The model under review builds one solid part; all positions refer to its coordinate system, in mm. A direction names the side the tool comes from. Coordinates: 2 decimals unless noted, no trailing zeros. Write each loop counter-clockwise with the first axis right and the second up, starting at its lowest first coordinate (ties: lowest second). Pieces come first, ordered by that corner, then holes.
```python
from build123d import *

# Parameters (mm, degrees)
BOSS_EXTRUDE1_DEPTH     = 2000
CUT_EXTRUDE1_DEPTH      = 2002.124683772
CUT_EXTRUDE1_DEPTH_BACK = 2002.124683772


with BuildPart() as part:
    # Sketch1 → Boss-Extrude1 (new body)
    with BuildSketch(Plane(origin=(0, 0, 0), x_dir=(1, 0, 0), z_dir=(0, 1, 0))):
        with BuildLine():
            Line((-20, -30), (20, -30))
            ThreePointArc((20, -30), (27.071067812, -27.071067812), (30, -20))
            Line((30, -20), (30, 20))
            ThreePointArc((30, 20), (27.071067812, 27.071067812), (20, 30))
            Line((20, 30), (-20, 30))
            ThreePointArc((-20, 30), (-27.071067812, 27.071067812), (-30, 20))
            Line((-30, 20), (-30, -20))
            ThreePointArc((-30, -20), (-27.071067812, -27.071067812), (-20, -30))
        make_face()
        with BuildLine():
            Line((-26, -20), (-26, 20))
            ThreePointArc((-26, 20), (-24.242640687, 24.242640687), (-20, 26))
            Line((-20, 26), (20, 26))
            ThreePointArc((20, 26), (24.242640687, 24.242640687), (26, 20))
            Line((26, 20), (26, -20))
            ThreePointArc((26, -20), (24.242640687, -24.242640687), (20, -26))
            Line((20, -26), (-20, -26))
            ThreePointArc((-20, -26), (-24.242640687, -24.242640687), (-26, -20))
        make_face(mode=Mode.SUBTRACT)
    extrude(amount=BOSS_EXTRUDE1_DEPTH)

    # Sketch2 → Cut-Extrude1 (cut, two sides: drawn at the far end of the back side and taken through both)
    with BuildSketch(Plane.XY.offset(30).offset(-CUT_EXTRUDE1_DEPTH_BACK)):
        Polygon((30, 0), (-30, 75.027298751), (-170.24369385, -210.007574385), align=None)
        Polygon((-30, 1484.027298751), (30, 1409), (525.992052796, 1638.556238223), (8.977575366, 2080.626411119), (-421.015295507, 1818.362615914), align=None)
    extrude(amount=CUT_EXTRUDE1_DEPTH + CUT_EXTRUDE1_DEPTH_BACK, mode=Mode.SUBTRACT)


solid = part.part
```
Item 1: Mouldability with a two-part tool opening along X and no side actions: class faces 3 (the face through (0, 732, -30)), 4 (the face through (30, 695, 0)), 5 (the face through (0, 732, -26)) as pulls with the +X half, pulls with the -X half, needs draft (parallel to the pull), parting line crosses it, or undercut.
Solved:
face 3: needs draft
face 4: pulls with the +X half
face 5: undercut
Item 2: Take a section at B-B, the plane y = 126. Write out the cut boundary in (x, z), plus the area to 3 significant figures.
Solved:
outline: (-30, -20) arc R10 ccw to (-20, -30) - (20, -30) arc R10 ccw to (30, -20) - (30, 20) arc R10 ccw to (20, 30) - (-20, 30) arc R10 ccw to (-30, 20) - close; hole (-26, -20) arc R6 ccw to (-20, -26) - (20, -26) arc R6 ccw to (26, -20) - (26, 20) arc R6 ccw to (20, 26) - (-20, 26) arc R6 ccw to (-26, 20) - close
area: 841 mm2
Item 3: Take a section at C-C, the plane x = 5.5. Write out the cut boundary in (y, z).
Solved:
outline: (30.64, -30) - (1439.64, -30) - (1439.64, -26) - (30.64, -26) - close; (30.64, 26) - (1439.64, 26) - (1439.64, 30) - (30.64, 30) - close
Item 4: Machinability: for faces 1 (the face through (0, 732, 26)), 2 (the face through (-0.42, 1447.04, 26.25)), which of the approach directions +Z, -Z, +X, -X, +Y, -Y give a long, thin tool a straight path to every point of the face, cutting with its end or side? Answer none if there is none.
Solved:
face 1: +Y, -Y
face 2: +Z, -Z, +X, +Y
Item 5: Take a section at A-A, the plane z = -0.5. Write out the cut boundary in (x, y), plus the area to 3 significant figures.
Solved:
outline: (-30, 75.03) - (-26, 70.03) - (-26, 1479.03) - (-30, 1484.03) - close; (26, 5) - (30, 0) - (30, 1409) - (26, 1414) - close
area: 11,300 mm2
Item 6: To check wall thickness, follow line 1 along Z through (x, y) = (-6.5, 1070); line 2 along Z through (x, y) = (-21, 841). State the ranges of each line that lie inside material, in increasing order.
Solved:
line 1: z = -30 to -26, 26 to 30
line 2: z = -29.95 to -25.92, 25.92 to 29.95
